from build123d import *

# Parameters (mm, degrees)
SKETCH_1_R          = 21
SKETCH_1_R_2        = 14.575
SKETCH_1_R_3        = 23.75
SKETCH_1_R_4        = 2.1
SKETCH_1_R_5        = 3
EXTRUDE_1_DEPTH     = 10
CUT_EXTRUDE_1_DEPTH = 10
FILLET_1_R          = 20
CUT_EXTRUDE_2_DEPTH = 10
FILLET_2_R          = 5
SKETCH_5_R          = 3
CUT_EXTRUDE_3_DEPTH = 10
CUT_EXTRUDE_5_DEPTH = 10


with BuildPart() as part:
    # 草图1 → 凸台-拉伸1 (new body)
    with BuildSketch(Plane(origin=(0, 0, 0), x_dir=(1, 0, 0), z_dir=(0, 1, 0))):
        with BuildLine():
            Line((0, 27), (96.94985335, 27))
            ThreePointArc((96.94985335, 27), (104.319003455, 25.974903787), (111.128591496, 22.977453832))
            Line((111.128591496, 22.977453832), (137.853241587, 6.486426651))
            ThreePointArc((137.853241587, 6.486426651), (139.604326734, 5.629209592), (141.488462469, 5.12805811))
            Line((141.488462469, 5.12805811), (294.137288277, -19.871137584))
            ThreePointArc((294.137288277, -19.871137584), (320.161534926, -58.578669293), (279.908528522, -82.141986125))
            Line((279.908528522, -82.141986125), (257.295172569, -75.46881036))
            ThreePointArc((257.295172569, -75.46881036), (248.237976105, -77.886212941), (241.944328029, -70.938793499))
            Line((241.944328029, -70.938793499), (95.820417973, -27.817792917))
            ThreePointArc((95.820417973, -27.817792917), (93.01947824, -27.205504027), (90.159770359, -27))
            Line((90.159770359, -27), (0, -27))
            ThreePointArc((0, -27), (-27, 0), (0, 27))
        make_face()
        with Locations(Location((0, 0, 0), (0, 0, 270))):
            Circle(SKETCH_1_R, mode=Mode.SUBTRACT)
        with Locations(Location((96.94985335, 0, 0), (0, 0, 270))):
            Circle(SKETCH_1_R_2, mode=Mode.SUBTRACT)
        with Locations(Location((288.965564705, -51.450454792, 0), (0, 0, 270))):
            Circle(SKETCH_1_R_3, mode=Mode.SUBTRACT)
        with Locations(Location((288.965564705, -23.700454792, 0), (0, 0, 270))):
            Circle(SKETCH_1_R_4, mode=Mode.SUBTRACT)
        with Locations(Location((312.99776966, -37.575454792, 0), (0, 0, 270))):
            Circle(SKETCH_1_R_4, mode=Mode.SUBTRACT)
        with Locations(Location((312.99776966, -65.325454792, 0), (0, 0, 270))):
            Circle(SKETCH_1_R_4, mode=Mode.SUBTRACT)
        with Locations(Location((288.965564705, -79.200454792, 0), (0, 0, 270))):
            Circle(SKETCH_1_R_4, mode=Mode.SUBTRACT)
        with Locations(Location((264.93335975, -65.325454792, 0), (0, 0, 270))):
            Circle(SKETCH_1_R_4, mode=Mode.SUBTRACT)
        with Locations(Location((264.93335975, -37.575454792, 0), (0, 0, 270))):
            Circle(SKETCH_1_R_4, mode=Mode.SUBTRACT)
        with Locations(Location((250.785267532, -69.254219754, 0), (0, 0, 270))):
            Circle(SKETCH_1_R_5, mode=Mode.SUBTRACT)
    extrude(amount=EXTRUDE_1_DEPTH)

    # 草图3 → 切除-拉伸1 (cut)
    with BuildSketch(Plane(origin=(0, 10, 0), x_dir=(1, 0, 0), z_dir=(0, 1, 0))):
        with BuildLine():
            Line((243.704770173, -111.253970394), (131.873115991, -26.616980894))
            ThreePointArc((131.873115991, -26.616980894), (128.702921113, -25.009854291), (125.170844375, -24.613085592))
            Line((125.170844375, -24.613085592), (88.824772335, -27.044605234))
            Line((88.824772335, -27.044605234), (243.704770173, -111.253970394))
        make_face()
    extrude(amount=-CUT_EXTRUDE_1_DEPTH, mode=Mode.SUBTRACT)

    # 圆角1
    fillet_1_edges = [part.edges().sort_by_distance(p)[0] for p in [
        (257.295172569, 5, 75.46881036),
        (241.944328029, 5, 70.938793499),
        (157.515855554, 5, 46.024046766),
    ]]
    fillet(fillet_1_edges, radius=FILLET_1_R)

    # 草图4 → 切除-拉伸2 (cut)
    with BuildSketch(Plane(origin=(0, 10, 0), x_dir=(1, 0, 0), z_dir=(0, 1, 0))):
        with BuildLine():
            ThreePointArc((73.530936261, -7.448821877), (73.010770558, 5.554362258), (79.203568528, 17))
            Line((79.203568528, 17), (35.21775864, 17))
            Line((35.21775864, 17), (73.530936261, -7.448821877))
        make_face()
        with BuildLine():
            Line((69.908772681, -17), (29.781319723, 8.606567001))
            ThreePointArc((29.781319723, 8.606567001), (30.653969418, -4.618891526), (25.922962794, -17))
            Line((25.922962794, -17), (69.908772681, -17))
        make_face()
        with BuildLine():
            Line((218.588169342, -17.631723767), (252.130615229, -59.711749917))
            ThreePointArc((252.130615229, -59.711749917), (252.70586007, -40.94824932), (262.247669453, -24.781810782))
            Line((262.247669453, -24.781810782), (218.588169342, -17.631723767))
        make_face()
        Polygon((139.872298853, -4.740478518), (229.34372575, -56.794041123), (195.054934366, -13.777701679), align=None)
    extrude(amount=-CUT_EXTRUDE_2_DEPTH, mode=Mode.SUBTRACT)

    # 圆角2
    fillet_2_edges = [part.edges().sort_by_distance(p)[0] for p in [
        (25.922962794, 5, 17),
        (29.781319723, 5, -8.606567001),
        (69.908772681, 5, 17),
        (139.872298853, 5, 4.740478518),
        (195.054934366, 5, 13.777701679),
        (229.34372575, 5, 56.794041123),
        (262.247669453, 5, 24.781810782),
        (252.130615229, 5, 59.711749917),
        (218.588169342, 5, 17.631723767),
        (79.203568528, 5, -17),
        (73.530936261, 5, 7.448821877),
        (35.21775864, 5, -17),
    ]]
    fillet(fillet_2_edges, radius=FILLET_2_R)

    # 草图5 → 切除-拉伸3 (cut)
    with BuildSketch(Plane(origin=(0, 10, 0), x_dir=(1, 0, 0), z_dir=(0, 1, 0))):
        with Locations(Location((205.845927584, -15.544935392, 0), (0, 0, 270))):
            Circle(SKETCH_5_R)
    extrude(amount=-CUT_EXTRUDE_3_DEPTH, mode=Mode.SUBTRACT)

    # 草图7 → 切除-拉伸5 (cut)
    with BuildSketch(Plane.XZ):
        with BuildLine():
            Line((171.32105295, 38.077089469), (188.608233051, 48.134594337))
            ThreePointArc((188.608233051, 48.134594337), (192.709935796, 47.050143053), (191.625484511, 42.948440307))
            Line((191.625484511, 42.948440307), (174.338304411, 32.890935439))
            ThreePointArc((174.338304411, 32.890935439), (170.236601666, 33.975386724), (171.32105295, 38.077089469))
        make_face()
    extrude(amount=-CUT_EXTRUDE_5_DEPTH, mode=Mode.SUBTRACT)


solid = part.part
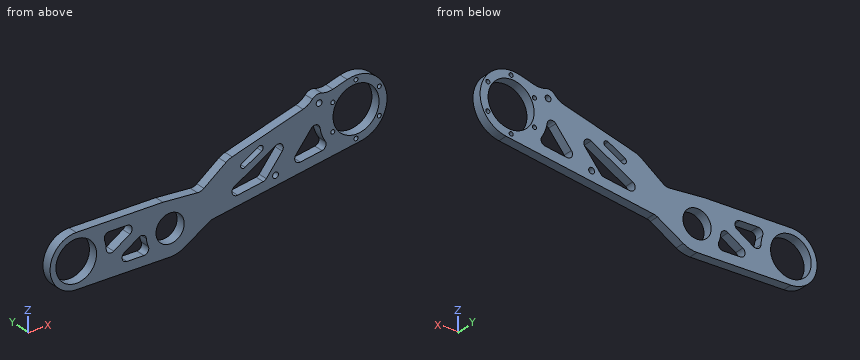
Part model, mm, in its own coordinate system. Give positions to 0.01 mm unless a question says otherwise; leave off trailing zeros. Loops run counter-clockwise (first coordinate to the right, second up) from the corner with the lowest first, then second, coordinate; pieces in that order, holes last. Notation, with made-up numbers: (-36, 85) -> (-22, 85) arc R8 cw to (-22, 98) -> close; hole circle Ø10 at (61.25, 71). An arc over 180 degrees is marked (long way). Write each question's results on one line, items separated by ' | '. Start each with the question number.
Q1. Wall check: L1, parallel to Z at x = 264, y = 4.25; L2, parallel to Z at x = 45, y = 1.75; L3, parallel to Z at x = 290, y = 8.25. Give the ranges that are in metal, low to high.
Q2. Band-saw the part on C-C on y = 5. Count the separate pieces of the cut face and the enclosed holes in it, plus the area to 3 significant figures.
Q3. Band-saw the part on B-B on x = 86. List the corners of the cut face in (y, z), plus the area to 3 significant figures.
Q4. Band-saw the part on A-A on z = 57.5. List the corners of the cut face in (x, y), plus the area to 3 significant figures.
Q5. Pin check, flat tips, straight feed: P1, Ø4, axis at y = 5, z = 6.5, coming from the -X side; P2, Ø3, axis at x = 57, y = 5.5, coming from the +Z side; P3, Ø2, axis at y = 1, z = 36, coming from the +X side. Stop position of each tip, or through.
Results are:
1) L1: z = 14.94 to 35.69, 39.46 to 63.44, 67.21 to 77.48 | L2: z = -27 to 1.1, 17 to 27 | L3: z = 19.19 to 21.87, 25.53 to 27.72, 75.18 to 77.37, 81.03 to 83.43
2) separate pieces: 1 | enclosed holes: 16 | area: 11,900 mm²
3) outline: (0, -27) -> (10, -27) -> (10, -9.62) -> (0, -9.62) -> close; (0, 9.62) -> (10, 9.62) -> (10, 27) -> (0, 27) -> close | area: 348 mm²
4) outline: (196.4, 0) -> (266, 0) -> (266, 10) -> (196.4, 10) -> close; (311.93, 0) -> (320.39, 0) -> (320.39, 10) -> (311.93, 10) -> close | area: 781 mm²
5) P1: stops at x = -26.62 | P2: stops at z = 27 | P3: stops at x = 317.52
